```python
from build123d import *

# Parameters (mm, degrees)
SKETCH_1_W          = 88.5
SKETCH_1_H          = 46
SKETCH_1_R          = 1.6
EXTRUDE_1_DEPTH     = 2
CUT_EXTRUDE_1_DEPTH = 50.910544978
FILLET_1_R          = 2


with BuildPart() as part:
    # 草图1 → 凸台-拉伸1 (new body)
    with BuildSketch(Plane(origin=(0, 0, 0), x_dir=(1, 0, 0), z_dir=(0, 1, 0))):
        Rectangle(SKETCH_1_W, SKETCH_1_H)
        with Locations(Location((-41.25, -5.5, 0), (0, 0, 270))):
            Circle(SKETCH_1_R, mode=Mode.SUBTRACT)
        with Locations(Location((-41.25, -15.5, 0), (0, 0, 270))):
            Circle(SKETCH_1_R, mode=Mode.SUBTRACT)
        with Locations(Location((41.25, -15.5, 0), (0, 0, 90))):
            Circle(SKETCH_1_R, mode=Mode.SUBTRACT)
        with Locations(Location((41.25, -5.5, 0), (0, 0, 90))):
            Circle(SKETCH_1_R, mode=Mode.SUBTRACT)
        with Locations(Location((-8.75, -20, 0), (0, 0, 270))):
            Circle(SKETCH_1_R, mode=Mode.SUBTRACT)
        with Locations(Location((1.25, -20, 0), (0, 0, 270))):
            Circle(SKETCH_1_R, mode=Mode.SUBTRACT)
        with Locations(Location((-31, 17, 0), (0, 0, 270))):
            Circle(SKETCH_1_R, mode=Mode.SUBTRACT)
        with Locations(Location((-18, 17, 0), (0, 0, 270))):
            Circle(SKETCH_1_R, mode=Mode.SUBTRACT)
        with Locations(Location((18, 17, 0), (0, 0, 270))):
            Circle(SKETCH_1_R, mode=Mode.SUBTRACT)
        with Locations(Location((31, 17, 0), (0, 0, 270))):
            Circle(SKETCH_1_R, mode=Mode.SUBTRACT)
    extrude(amount=EXTRUDE_1_DEPTH)

    # 草图2 → 切除-拉伸1 (cut, through all)
    with BuildSketch(Plane(origin=(0, 2, 0), x_dir=(1, 0, 0), z_dir=(0, 1, 0))):
        with BuildLine():
            Line((-27.75, 10), (-27.75, -13))
            ThreePointArc((-27.75, -13), (-31.25, -16.5), (-34.75, -13))
            Line((-34.75, -13), (-34.75, 10))
            ThreePointArc((-34.75, 10), (-31.25, 13.5), (-27.75, 10))
        make_face()
        with BuildLine():
            Line((-15.25, 10), (-15.25, -13))
            ThreePointArc((-15.25, -13), (-18.75, -16.5), (-22.25, -13))
            Line((-22.25, -13), (-22.25, 10))
            ThreePointArc((-22.25, 10), (-18.75, 13.5), (-15.25, 10))
        make_face()
        with BuildLine():
            Line((-2.75, 10), (-2.75, -13))
            ThreePointArc((-2.75, -13), (-6.25, -16.5), (-9.75, -13))
            Line((-9.75, -13), (-9.75, 10))
            ThreePointArc((-9.75, 10), (-6.25, 13.5), (-2.75, 10))
        make_face()
        with BuildLine():
            Line((9.75, 10), (9.75, -13))
            ThreePointArc((9.75, -13), (6.25, -16.5), (2.75, -13))
            Line((2.75, -13), (2.75, 10))
            ThreePointArc((2.75, 10), (6.25, 13.5), (9.75, 10))
        make_face()
        with BuildLine():
            Line((22.25, 10), (22.25, -13))
            ThreePointArc((22.25, -13), (18.75, -16.5), (15.25, -13))
            Line((15.25, -13), (15.25, 10))
            ThreePointArc((15.25, 10), (18.75, 13.5), (22.25, 10))
        make_face()
        with BuildLine():
            Line((34.75, 10), (34.75, -13))
            ThreePointArc((34.75, -13), (31.25, -16.5), (27.75, -13))
            Line((27.75, -13), (27.75, 10))
            ThreePointArc((27.75, 10), (31.25, 13.5), (34.75, 10))
        make_face()
        with BuildLine():
            Line((-11, 20), (11, 20))
            ThreePointArc((11, 20), (13, 18), (11, 16))
            Line((11, 16), (-11, 16))
            ThreePointArc((-11, 16), (-13, 18), (-11, 20))
        make_face()
    extrude(amount=-CUT_EXTRUDE_1_DEPTH, mode=Mode.SUBTRACT)

    # 圆角1
    fillet_1_edges = [part.edges().sort_by_distance(p)[0] for p in [
        (44.25, 1, 23),
        (-44.25, 1, 23),
        (-44.25, 1, -23),
        (44.25, 1, -23),
    ]]
    fillet(fillet_1_edges, radius=FILLET_1_R)


solid = part.part
```
Part model, mm, in its own coordinate system. A direction names the side the tool comes from. Round coordinates to 2 decimals unless told otherwise and drop trailing zeros. Write each loop counter-clockwise with the first axis right and the second up, starting at its lowest first coordinate (ties: lowest second). Pieces come first, ordered by that corner, then holes. Notation, with made-up numbers: (82, 2) -> (125, 2) arc R28 ccw to (125, 33) -> close; hole circle Ø5 at (-21, 2.25). An arc over 180 degrees is marked (long way). Return JSON: item names as keys, results as strings. Group by question number.
Q1. Pin check, flat tip, straight feed: pin 1 (1.9 mm diameter, centred on x = 1.25, z = 20, fed in from -Y). Stop position of the tip, or through.
Q2. Saw through at B-B on z = 1.5. Write the cut outline in (x, y), plus the area to 3 significant figures.
Q3. Saw through at A-A on x = 1.25. Write the cut outline in (y, z), plus the area to 3 significant figures.
Q4. Mould opens along X. For faces 3 (the flat face through (-1, 2, 0)), 4 (the cylindrical face through (-43.68, 1.01, -22.4)), 5 (the flat face through (2.75, 1, 2)) say: pulls with the +X half, pulls with the -X half, needs draft (parallel to the pull), parting line crosses it, or undercut.
Q5. Which spindle directions (+Z, -Z, +X, -X, +Y, -Y) get a long thin tool onto all of the face, cutting with end or side? Do faces 1 (the cylindrical face through (43.65, 1.01, -22.43)), 2 (the flat face through (22.25, 1, 1)). Say none if no direction does.
Q6. Saw through at C-C on x = -8.75. Write the cut outline in (y, z), plus the area to 3 significant figures.
Q7. Saw through at D-D on y = 1.45. State how many separate pieces and enclosed holes the cut face has, plus the area to 3 significant figures.
Q8. Probe L1, parallel to Z at x = 11, y = 0.7; L2, parallel to Z at x = 12, y = 0.3. List the from-to ranges inside material, lowest first. Write a range as [from, to].
Answer:
{
 "1": {"pin 1": "through"},
 "2": {"outline": "(-44.25, 0) -> (-34.75, 0) -> (-34.75, 2) -> (-44.25, 2) -> close; (-27.75, 0) -> (-22.25, 0) -> (-22.25, 2) -> (-27.75, 2) -> close; (-15.25, 0) -> (-9.75, 0) -> (-9.75, 2) -> (-15.25, 2) -> close; (-2.75, 0) -> (2.75, 0) -> (2.75, 2) -> (-2.75, 2) -> close; (9.75, 0) -> (15.25, 0) -> (15.25, 2) -> (9.75, 2) -> close; (22.25, 0) -> (27.75, 0) -> (27.75, 2) -> (22.25, 2) -> close; (34.75, 0) -> (44.25, 0) -> (44.25, 2) -> (34.75, 2) -> close", "area": "93.0 mm2"},
 "3": {"outline": "(0, -23) -> (2, -23) -> (2, -20) -> (0, -20) -> close; (0, -16) -> (2, -16) -> (2, 18.4) -> (0, 18.4) -> close; (0, 21.6) -> (2, 21.6) -> (2, 23) -> (0, 23) -> close", "area": "77.6 mm2"},
 "4": {"face 3": "needs draft", "face 4": "pulls with the -X half", "face 5": "undercut"},
 "5": {"face 1": "-Z, +X, +Y, -Y", "face 2": "+Y, -Y"},
 "6": {"outline": "(0, -23) -> (2, -23) -> (2, -20) -> (0, -20) -> close; (0, -16) -> (2, -16) -> (2, -12.45) -> (0, -12.45) -> close; (0, 15.45) -> (2, 15.45) -> (2, 18.4) -> (0, 18.4) -> close; (0, 21.6) -> (2, 21.6) -> (2, 23) -> (0, 23) -> close", "area": "21.8 mm2"},
 "7": {"separate pieces": "1", "enclosed holes": "17", "area": "2,690 mm2"},
 "8": {"L1": "[-23, -20], [-16, 23]", "L2": "[-23, -19.73], [-16.27, 23]"}
}
